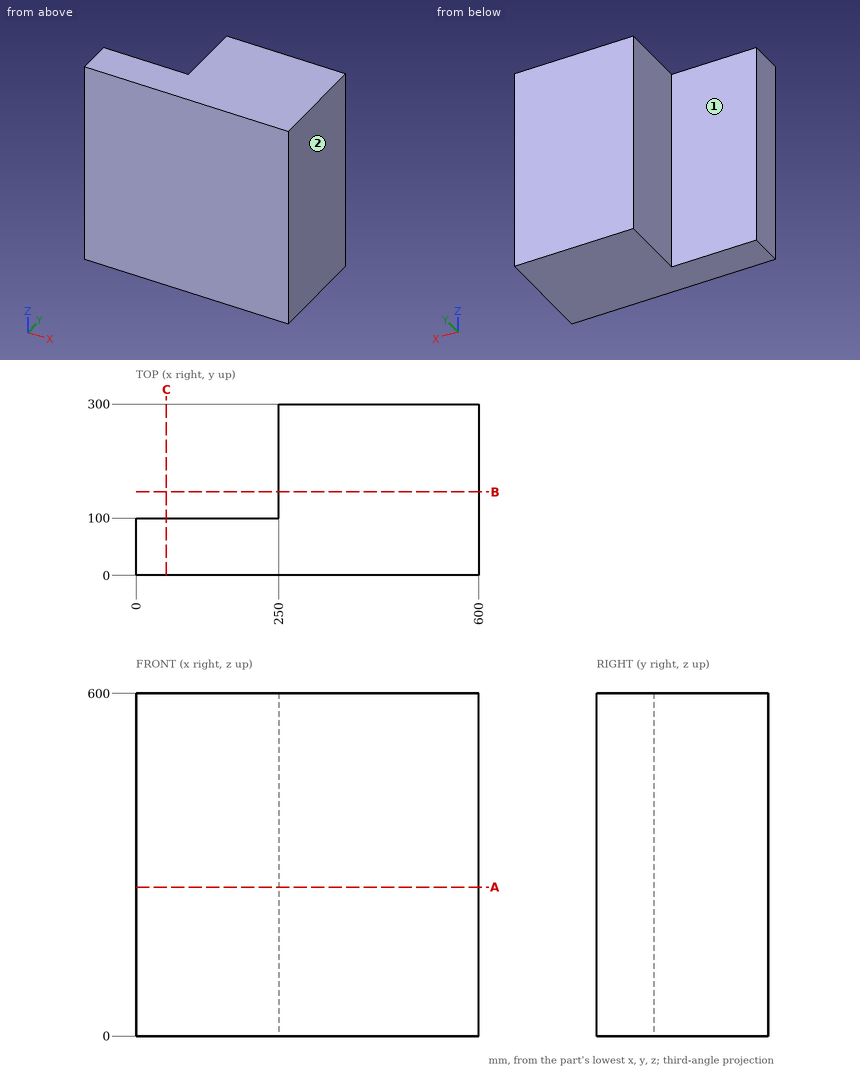
Design review of the part shown in the three views and the two pictorial views. Dimensions are in mm from the part's minimum x, y and z. A direction names the side the tool comes from. Round coordinates to 2 decimals unless told otherwise and drop trailing zeros. Loops run counter-clockwise (first coordinate to the right, second up) from the corner with the lowest first, then second, coordinate; pieces in that order, holes last.
1) Consider section A-A on z = 260.5. State the section outline as (x, y) points.
Values follow:
outline: (0, 0) - (600, 0) - (600, 300) - (250, 300) - (250, 100) - (0, 100) - close
2) Consider section C-C on x = 53. State the section outline as (y, z) points, then the cut area to 3 significant figures.
Values follow:
outline: (0, 0) - (100, 0) - (100, 600) - (0, 600) - close
area: 60,000 mm2
3) Tool access review of the marked faces 1 and 2: name each direction out of +Z, -Z, +X, -X, +Y, -Y from which nothing blocks a thin tool from reaching the whole face with its end or side.
Values follow:
face 1: +Z, -Z, -X, +Y
face 2: +Z, -Z, +X, +Y, -Y
4) Consider section B-B on y = 146. State the section outline as (x, z) points.
Values follow:
outline: (250, 0) - (600, 0) - (600, 600) - (250, 600) - close
5) Clearance check with flat-ended pins moving along their axes: P1, Ø8, axis at y = 132, z = 491, coming from the -X side; P2, Ø5, axis at y = 76, z = 113, coming from the -X side. State where each tip first meets the part, or that it passes through.
Values follow:
P1: stops at x = 250
P2: stops at x = 0
6) Wall thickness on line 1 along X through (y, z) = (201.5, 460); line 2 along Y through (x, z) = (166.5, 185): over which ranges is each line inside the solid? List them lowest first.
Values follow:
line 1: x = 250 to 600
line 2: y = 0 to 100
